The listing builds one solid part. Answer for the finished solid, in the listing's coordinates (mm). A direction names the side the tool comes from. Round coordinates to 2 decimals unless told otherwise and drop trailing zeros. Write each loop counter-clockwise with the first axis right and the second up, starting at its lowest first coordinate (ties: lowest second). Pieces come first, ordered by that corner, then holes. Notation, with made-up numbers: M -4,43.5 L 47,43.5 A23 cw 47,79.5 Z; hole C 78,22 d3. An arc over 180 degrees is marked long. Write each question's results on one line, items separated by ' | '.
from build123d import *

# Parameters (mm, degrees)
SKETCH_1_W          = 136
SKETCH_1_H          = 46
SKETCH_1_R          = 1.6
EXTRUDE_1_DEPTH     = 2
CUT_EXTRUDE_1_DEPTH = 72.812255222
FILLET_R2_1_R       = 2


with BuildPart() as part:
    # 草图1 → 凸台-拉伸1 (new body)
    with BuildSketch(Plane(origin=(0, 0, 0), x_dir=(1, 0, 0), z_dir=(0, 1, 0))):
        Rectangle(SKETCH_1_W, SKETCH_1_H)
        with Locations(Location((-63, -0.5, 0), (0, 0, 270))):
            Circle(SKETCH_1_R, mode=Mode.SUBTRACT)
        with Locations(Location((-63, -10.5, 0), (0, 0, 270))):
            Circle(SKETCH_1_R, mode=Mode.SUBTRACT)
        with Locations(Location((-5, -20, 0), (0, 0, 270))):
            Circle(SKETCH_1_R, mode=Mode.SUBTRACT)
        with Locations(Location((5, -20, 0), (0, 0, 270))):
            Circle(SKETCH_1_R, mode=Mode.SUBTRACT)
        with Locations(Location((63, -10.5, 0), (0, 0, 90))):
            Circle(SKETCH_1_R, mode=Mode.SUBTRACT)
        with Locations(Location((63, -0.5, 0), (0, 0, 90))):
            Circle(SKETCH_1_R, mode=Mode.SUBTRACT)
        with Locations(Location((5, 20, 0), (0, 0, 90))):
            Circle(SKETCH_1_R, mode=Mode.SUBTRACT)
        with Locations(Location((-5, 20, 0), (0, 0, 90))):
            Circle(SKETCH_1_R, mode=Mode.SUBTRACT)
    extrude(amount=EXTRUDE_1_DEPTH)

    # 草图2 → 切除-拉伸1 (cut, through all)
    with BuildSketch(Plane(origin=(0, 2, 0), x_dir=(1, 0, 0), z_dir=(0, 1, 0))):
        with BuildLine():
            Line((-50.5, 15), (-50.5, -15))
            ThreePointArc((-50.5, -15), (-54, -18.5), (-57.5, -15))
            Line((-57.5, -15), (-57.5, 15))
            ThreePointArc((-57.5, 15), (-54, 18.5), (-50.5, 15))
        make_face()
        with BuildLine():
            Line((-38.5, 15), (-38.5, -15))
            ThreePointArc((-38.5, -15), (-42, -18.5), (-45.5, -15))
            Line((-45.5, -15), (-45.5, 15))
            ThreePointArc((-45.5, 15), (-42, 18.5), (-38.5, 15))
        make_face()
        with BuildLine():
            Line((-26.5, 15), (-26.5, -15))
            ThreePointArc((-26.5, -15), (-30, -18.5), (-33.5, -15))
            Line((-33.5, -15), (-33.5, 15))
            ThreePointArc((-33.5, 15), (-30, 18.5), (-26.5, 15))
        make_face()
        with BuildLine():
            Line((-14.5, 15), (-14.5, -15))
            ThreePointArc((-14.5, -15), (-18, -18.5), (-21.5, -15))
            Line((-21.5, -15), (-21.5, 15))
            ThreePointArc((-21.5, 15), (-18, 18.5), (-14.5, 15))
        make_face()
        with BuildLine():
            Line((-2.5, 12), (-2.5, -12))
            ThreePointArc((-2.5, -12), (-6, -15.5), (-9.5, -12))
            Line((-9.5, -12), (-9.5, 12))
            ThreePointArc((-9.5, 12), (-6, 15.5), (-2.5, 12))
        make_face()
        with BuildLine():
            Line((9.5, 12), (9.5, -12))
            ThreePointArc((9.5, -12), (6, -15.5), (2.5, -12))
            Line((2.5, -12), (2.5, 12))
            ThreePointArc((2.5, 12), (6, 15.5), (9.5, 12))
        make_face()
        with BuildLine():
            Line((21.5, 15), (21.5, -15))
            ThreePointArc((21.5, -15), (18, -18.5), (14.5, -15))
            Line((14.5, -15), (14.5, 15))
            ThreePointArc((14.5, 15), (18, 18.5), (21.5, 15))
        make_face()
        with BuildLine():
            Line((33.5, 15), (33.5, -15))
            ThreePointArc((33.5, -15), (30, -18.5), (26.5, -15))
            Line((26.5, -15), (26.5, 15))
            ThreePointArc((26.5, 15), (30, 18.5), (33.5, 15))
        make_face()
        with BuildLine():
            Line((45.5, 15), (45.5, -15))
            ThreePointArc((45.5, -15), (42, -18.5), (38.5, -15))
            Line((38.5, -15), (38.5, 15))
            ThreePointArc((38.5, 15), (42, 18.5), (45.5, 15))
        make_face()
        with BuildLine():
            Line((57.5, 15), (57.5, -15))
            ThreePointArc((57.5, -15), (54, -18.5), (50.5, -15))
            Line((50.5, -15), (50.5, 15))
            ThreePointArc((50.5, 15), (54, 18.5), (57.5, 15))
        make_face()
    extrude(amount=-CUT_EXTRUDE_1_DEPTH, mode=Mode.SUBTRACT)

    # R2 圆角1
    fillet_r2_1_edges = [part.edges().sort_by_distance(p)[0] for p in [
        (-68, 1, -23),
        (68, 1, -23),
        (68, 1, 23),
        (-68, 1, 23),
    ]]
    fillet(fillet_r2_1_edges, radius=FILLET_R2_1_R)


solid = part.part
1) Section C-C (z = 0.5) is taken. State how many separate pieces and enclosed holes the cut face has, then the cut area to 3 significant figures.
Return value:
separate pieces: 13 | enclosed holes: 0 | area: 119 mm²
2) Find the intervals of material crossed by line 1 (X direction, y = 1, z = 20); line 2 (X direction, y = 1, z = 20.5); line 3 (Z direction, x = 41.5, y = 0.5), in increasing order.
Return value:
line 1: -68 to -6.6, -3.4 to 3.4, 6.6 to 68 | line 2: -68 to -6.52, -3.48 to 3.48, 6.52 to 68 | line 3: -23 to -18.46, 18.46 to 23
3) Section A-A (x = -63) is taken. Determine the outline of the cut face in (y, z), then the cut area to 3 significant figures.
Return value:
outline: M 0,-23 L 2,-23 L 2,-1.1 L 0,-1.1 Z; M 0,2.1 L 2,2.1 L 2,8.9 L 0,8.9 Z; M 0,12.1 L 2,12.1 L 2,23 L 0,23 Z | area: 79.2 mm²
4) The mould has two halves that part along Z. Classify faces 1 (the face through (-1, 2, 0)), 2 (the face through (61.414, 0.986, 0.708)): +Z half, -Z half, draft (parallel to the pull), parting line (faces both ways), or undercut.
Return value:
face 1: draft | face 2: undercut
5) A tool of negligible diameter and unlimited length cuts with its end or side. For faces 3 (the face through (-1, 0, 0)), 4 (the face through (54.1, 1, 18.5)), from which of +Z, -Z, +X, -X, +Y, -Y can it reach the whole face along a straight path? Write none if from no direction.
Return value:
face 3: +Z, -Z, +X, -X, -Y | face 4: +Y, -Y
6) Section B-B (x = -42) is taken. Determine the outline of the cut face in (y, z), then the cut area to 3 significant figures.
Return value:
outline: M 0,-23 L 2,-23 L 2,-18.5 L 0,-18.5 Z; M 0,18.5 L 2,18.5 L 2,23 L 0,23 Z | area: 18.0 mm²
